```python
from build123d import *

# Parameters (mm, degrees)
BOSS_EXTRUDE1_DEPTH = 310
BOSS_EXTRUDE2_START = -26
SKETCH2_R           = 5
BOSS_EXTRUDE2_DEPTH = 55


with BuildPart() as part:
    # Sketch1 → Boss-Extrude1 (new, symmetric)
    with BuildSketch(Plane.XY):
        Polygon((0, 0), (7.5, 12.990381057), (0, 25.980762114), (0, 87.421161675), (-7.267949192, 100.009618943), (-0.200961894, 112.25), (-1.5, 113), (-9, 100.009618943), (-1.5, 87.019237886), (-1.5, 25.578838325), (5.767949192, 12.990381057), (-1.299038106, 0.75), align=None)
    extrude(amount=BOSS_EXTRUDE1_DEPTH, both=True)

    # Sketch2 → Boss-Extrude2 (add)
    with BuildSketch(Plane.XY.offset(310).offset(BOSS_EXTRUDE2_START)):
        with Locations((-0.75, 56.5)):
            Circle(SKETCH2_R)
    boss_extrude2 = extrude(amount=BOSS_EXTRUDE2_DEPTH)

    # Mirror1: Boss-Extrude2 across plane
    add(boss_extrude2.mirror(Plane.XY))


solid = part.part
```
Geometry: final body of the model. Coordinates: model frame, mm. Coordinates: 2 decimals unless noted, no trailing zeros. Order: outer loops, then holes, each group sorted by start corner. A loop starts at its lowest first (then second) coordinate and runs counter-clockwise, first axis right, second up. Notation, with made-up numbers: (45.25, -27) - (72.25, -27) arc R24 ccw to (72.25, -7) - close; hole circle Ø10 at (56, 15). An arc over 180 degrees is marked (long way). Return JSON: item names as keys, results as strings. Group by question number.
1. Material intervals for line 1 along X through (y, z) = (32.5, -81.5); line 2 along Y through (x, z) = (4, -203.5); line 3 along Y through (x, z) = (-6.25, -8), sorted ascending. Write a range as [from, to].
2. Pull-direction query (Y, two-part tool) for faces 1 (the face through (3.698, 6.404, 4.34)), 2 (the face through (-5.198, 106.596, 4.34)), 3 (the face through (-3.784, 106.044, 4.34)), 4 (the face through (-3.583, 93.627, 4.34)); classes: pulls with the +Y half, pulls with the -Y half, needs draft (parallel to the pull), parting line crosses it, or undercut.
3. Cut plane A-A (z = -104.5). Output: boundary loops of the cut face in (x, y), plus the area to 3 significant figures.
4. Pin query (flat end, axial travel): pin 1 (4.5 mm diameter, centred on x = 2, y = 36, fed in from -Z); pin 2 (18.5 mm diameter, centred on y = 45.5, z = 147, fed in from -X); pin 3 (10 mm diameter, centred on y = 56.5, z = -212.5, fed in from +X). Return the tip coordinate at first contact, or that it passes through.
Resolved:
{
 "1": {"line 1": "x = [-1.5, 0]", "line 2": "y = [6.93, 9.93], [16.05, 19.05]", "line 3": "y = [95.25, 98.25], [101.77, 104.77]"},
 "2": {"face 1": "pulls with the -Y half", "face 2": "pulls with the +Y half", "face 3": "undercut", "face 4": "undercut"},
 "3": {"outline": "(-9, 100.01) - (-1.5, 87.02) - (-1.5, 25.58) - (5.77, 12.99) - (-1.3, 0.75) - (0, 0) - (7.5, 12.99) - (0, 25.98) - (0, 87.42) - (-7.27, 100.01) - (-0.2, 112.25) - (-1.5, 113) - close", "area": "180 mm²"},
 "4": {"pin 1": "stops at z = -310", "pin 2": "stops at x = -1.5", "pin 3": "stops at x = 0"}
}
